from build123d import *
from OCP.BRepFilletAPI import BRepFilletAPI_MakeChamfer

# Parameters (mm, degrees)
SKETCH1_R        = 2.067
BASENUT_DEPTH    = 4.7
ENDCHAMFER_SIZE  = 0.433
ENDCHAMFER_SIZE2 = 0.249992667


with BuildPart() as part:
    # Sketch1 → BaseNut (new body)
    with BuildSketch(Plane.XY):
        Polygon((4.618802154, 0), (2.309401077, 4), (-2.309401077, 4), (-4.618802154, 0), (-2.309401077, -4), (2.309401077, -4), align=None)
        Circle(SKETCH1_R, mode=Mode.SUBTRACT)
    extrude(amount=-BASENUT_DEPTH)

    # Sketch2 → Double-Chamfer (revolve, cut)
    with BuildSketch(Plane(origin=(0, 0, 0), x_dir=(1, 0, 0), z_dir=(0, 1, 0))):
        Polygon((-4.618802154, 4.7), (-3.625, 4.7), (-4.618802154, 4.126228059), align=None)
        Polygon((-4.618802154, 0.573771941), (-4.618802154, 0), (-3.625, 0), align=None)
    revolve(axis=Axis((0, 0, -3.375940562), (0, 0, 1)), mode=Mode.SUBTRACT)

    # EndChamfer: one chamfer whose edges measure the first distance from different faces: ONE call of the kernel's chamfer builder (chamfer() names one face for all edges)
    endchamfer_edges_1 = [part.edges().sort_by_distance(p)[0] for p in [
        (-2.067, 0, -4.7),
    ]]
    endchamfer_side_1 = [part.faces().sort_by_distance(p)[0] for p in [
        (-2.067, 0, -2.35),
    ]]
    endchamfer_edges_2 = [part.edges().sort_by_distance(p)[0] for p in [
        (-2.067, 0, 0),
    ]]
    endchamfer_side_2 = [part.faces().sort_by_distance(p)[0] for p in [
        (3.522469517, 0, 0),
    ]]
    endchamfer = BRepFilletAPI_MakeChamfer(part.part.solid().wrapped)
    for e in endchamfer_edges_1:
        endchamfer.Add(ENDCHAMFER_SIZE, ENDCHAMFER_SIZE2, e.wrapped, endchamfer_side_1[0].wrapped)  # the first distance lies on this face
    for e in endchamfer_edges_2:
        endchamfer.Add(ENDCHAMFER_SIZE, ENDCHAMFER_SIZE2, e.wrapped, endchamfer_side_2[0].wrapped)  # the first distance lies on this face
    add(Compound.cast(endchamfer.Shape()), mode=Mode.REPLACE)


solid = part.part
Geometry check sheet. Reference: the model listing, model coordinates, mm. Coordinates: 2 decimals unless noted, no trailing zeros. Loops run counter-clockwise (first coordinate to the right, second up) from the corner with the lowest first, then second, coordinate; pieces in that order, holes last. Notation, with made-up numbers: (-12, 50) - (16, 50) arc R18 cw to (16, 58) - close; hole circle Ø1 at (54, 72). An arc over 180 degrees is marked (long way). Use one line per item in the form item = value. Start each with the question number.
Item 1: Section check B-B, the plane z = -3.9. Enter the section's corners in (x, y), and give its area (3 significant figures).
Item 2: Mould release check, pull along Y, two halves, no side actions. Record for faces 1 (the face through (-0.9, 2.5, 0)), 2 (the face through (0, -4, -2)), 3 (the face through (-1.64, -1.26, -2.23)), 4 (the face through (3.48, 1.97, -2.32)): +Y half, -Y half, draft (parallel to the pull), parting line (faces both ways), or undercut.
Item 3: Thickness scan on probe 1 along Y at (x, z) = (0, -0.65); probe 2 along X at (y, z) = (-1.5, -4.1); probe 3 along Y at (x, z) = (0.75, -2.05). Record the ranges inside material, lowest first.
Item 4: Gauge pin test, flat ends, axial feed: pin 1 (2 mm diameter, centred on y = -0.5, z = -2, fed in from -X); pin 2 (2 mm diameter, centred on y = 1.5, z = -2.5, fed in from -X). Record the tip position at first contact, or that the pin passes through.
Computed:
q1.outline = (-4.62, 0) - (-2.31, -4) - (2.31, -4) - (4.62, 0) - (2.31, 4) - (-2.31, 4) - close; hole circle Ø4.13 at (0, 0)
q1.area = 42.0 mm2
q2.face_1 = draft
q2.face_2 = -Y half
q2.face_3 = undercut
q2.face_4 = +Y half
q3.probe_1 = -4 to -2.07, 2.07 to 4
q3.probe_2 = -3.75 to -1.42, 1.42 to 3.75
q3.probe_3 = -4 to -1.93, 1.93 to 4
q4.pin_1 = -4.62
q4.pin_2 = -4.33
